Part print with two shaded views. Sizes in mm from the minimum x, y, z corner. A direction names the side the tool comes from. Round coordinates to 2 decimals unless told otherwise and drop trailing zeros. Order: outer loops, then holes, each group sorted by start corner. A loop starts at its lowest first (then second) coordinate and runs counter-clockwise, first axis right, second up. Notation, with made-up numbers: (44, -25) -> (62, -25) arc R16 ccw to (62, -6) -> close; hole circle Ø8 at (71.5, 80.5). An arc over 180 degrees is marked (long way). Use a Markdown table: item, result. Add a question column.
Item 1: Slice it at B-B, the plane y = 36.5. Give the cut face in (x, z).
Item 2: Slice it at C-C, the plane x = 58.5. Give the cut face in (y, z).
Item 3: 3-axis set-ups, long thin cutter, end or side, ignore diameter. For the marked faces 1, 2 and 3: which of +Z, -Z, +X, -X, +Y, -Y reach the whole face in a straight line?
Item 4: Probe L1, parallel to Z at x = 16, y = 22; L2, parallel to X at y = 38, z = 31; L3, parallel to Y at x = 38, z = 7.5. List the from-to ranges inside material, lowest first.
Item 5: Slice it at D-D, the plane z = 3. Give the cut face in (x, y).
Item 6: Two-plate mould, pull along Y, no slides. Class the marked faces 4, 5, 6 and 7: released by +Y, released by -Y, zero draft, split by the parting line, or undercut.
Item 7: Slice it at A-A, the plane x = 38. Give the cut face in (y, z), plus the area to 3 significant figures.
Item 8: Pin check, flat tips, straight feed: pin 1 (13.5 mm diameter, centred on x = 43.5, y = 49, fed in from +Z); pin 2 (12 mm diameter, centred on y = 50, z = 37.5, fed in from -X); pin 3 (5 mm diameter, centred on y = 63.5, z = 23, fed in from -X). Stop position of each tip, or through.
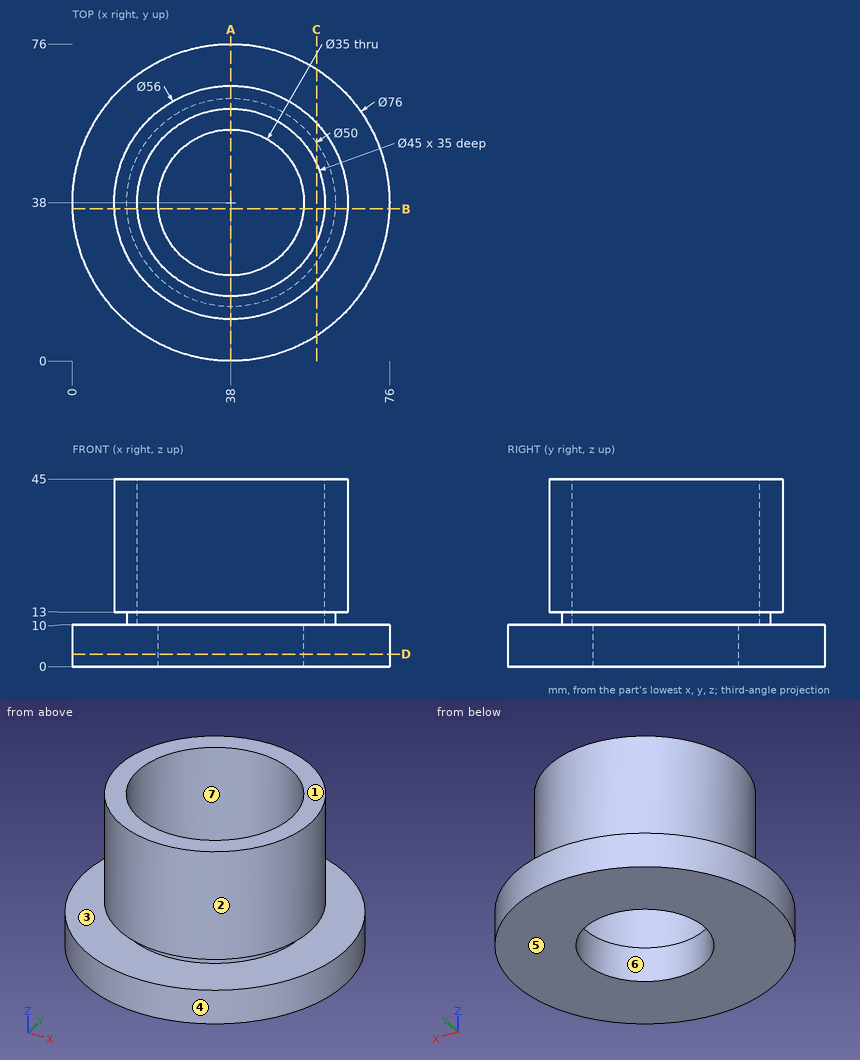
Check sheet entries:
| question | item | result |
|---|---|---|
| 1 | outline | (0.03, 0) -> (20.56, 0) -> (20.56, 10) -> (15.55, 10) -> (15.55, 45) -> (10.04, 45) -> (10.04, 13) -> (13.05, 13) -> (13.05, 10) -> (0.03, 10) -> close; (55.44, 0) -> (75.97, 0) -> (75.97, 10) -> (62.95, 10) -> (62.95, 13) -> (65.96, 13) -> (65.96, 45) -> (60.45, 45) -> (60.45, 10) -> (55.44, 10) -> close |
| 2 | outline | (6, 0) -> (70, 0) -> (70, 10) -> (52.31, 10) -> (52.31, 13) -> (57.07, 13) -> (57.07, 45) -> (47.27, 45) -> (47.27, 10) -> (28.73, 10) -> (28.73, 45) -> (18.93, 45) -> (18.93, 13) -> (23.69, 13) -> (23.69, 10) -> (6, 10) -> close |
| 3 | face 1 | +Z, +X, -X, +Y, -Y |
| 3 | face 2 | +Z |
| 3 | face 3 | none |
| 4 | L1 | 0 to 10, 13 to 45 |
| 4 | L2 | 10 to 15.5, 60.5 to 66 |
| 4 | L3 | 0 to 20.5, 55.5 to 76 |
| 5 | outline | circle Ø76 at (38, 38); hole circle Ø35 at (38, 38) |
| 6 | face 4 | split by the parting line |
| 6 | face 5 | zero draft |
| 6 | face 6 | undercut |
| 6 | face 7 | undercut |
| 7 | outline | (0, 0) -> (20.5, 0) -> (20.5, 10) -> (15.5, 10) -> (15.5, 45) -> (10, 45) -> (10, 13) -> (13, 13) -> (13, 10) -> (0, 10) -> close; (55.5, 0) -> (76, 0) -> (76, 10) -> (63, 10) -> (63, 13) -> (66, 13) -> (66, 45) -> (60.5, 45) -> (60.5, 10) -> (55.5, 10) -> close |
| 7 | area | 777 mm2 |
| 8 | pin 1 | z = 10 |
| 8 | pin 2 | x = 10.65 |
| 8 | pin 3 | x = 22.03 |
